Design review of the part built by this model. Coordinates are the model's own, in mm. Face numbers are marked on the shaded views. A direction names the side the tool comes from. Give positions to 0.01 mm unless a question says otherwise; leave off trailing zeros. Write each loop counter-clockwise with the first axis right and the second up, starting at its lowest first coordinate (ties: lowest second). Pieces come first, ordered by that corner, then holes. Notation, with made-up numbers: (29, 69) -> (60, 69) arc R13 cw to (60, 88) -> close; hole circle Ø3 at (23, -39). An arc over 180 degrees is marked (long way). Answer as a JSON object with one key per item and string values.
```python
from build123d import *

# Parameters (mm, degrees)
SKETCH_1_W               = 64
SKETCH_1_H               = 170
EXTRUDE_1_DEPTH          = 35
SKETCH_3_W               = 32.5
SKETCH_3_H               = 35
CUT_EXTRUDE_1_DEPTH      = 30
SKETCH_4_W               = 32.5
SKETCH_4_H               = 35
CUT_EXTRUDE_2_DEPTH      = 30
CUT_EXTRUDE_3_DEPTH      = 98.334474879
CUT_EXTRUDE_3_DEPTH_BACK = 98.334474879
SKETCH_5_R               = 5.5


with BuildPart() as part:
    # 草图1 → 凸台-拉伸1 (new body)
    with BuildSketch(Plane.XY):
        Rectangle(SKETCH_1_W, SKETCH_1_H)
    extrude(amount=EXTRUDE_1_DEPTH)

    # 草图3 → 切除-拉伸1 (cut)
    with BuildSketch(Plane.XY.offset(35)):
        with Locations((15.75, 67.5)):
            Rectangle(SKETCH_3_W, SKETCH_3_H)
        with Locations((15.75, -67.5)):
            Rectangle(SKETCH_3_W, SKETCH_3_H)
    extrude(amount=-CUT_EXTRUDE_1_DEPTH, mode=Mode.SUBTRACT)

    # 草图4 → 切除-拉伸2 (cut)
    with BuildSketch(Plane(origin=(0, 0, 0), x_dir=(-1, 0, 0), z_dir=(0, 0, -1))):
        with Locations((15.75, 67.5)):
            Rectangle(SKETCH_4_W, SKETCH_4_H)
        with Locations((15.75, -67.5)):
            Rectangle(SKETCH_4_W, SKETCH_4_H)
    extrude(amount=-CUT_EXTRUDE_2_DEPTH, mode=Mode.SUBTRACT)

    # 草图5 → 切除-拉伸3 (cut, two sides: drawn at the far end of the back side and taken through both)
    with BuildSketch(Plane.XY.offset(35).offset(-CUT_EXTRUDE_3_DEPTH_BACK)):
        with Locations((-18, 75)):
            Circle(SKETCH_5_R)
        with Locations((18, 75)):
            Circle(SKETCH_5_R)
        with Locations((18, -75)):
            Circle(SKETCH_5_R)
        with Locations((-18, -75)):
            Circle(SKETCH_5_R)
    extrude(amount=CUT_EXTRUDE_3_DEPTH + CUT_EXTRUDE_3_DEPTH_BACK, mode=Mode.SUBTRACT)


solid = part.part
```
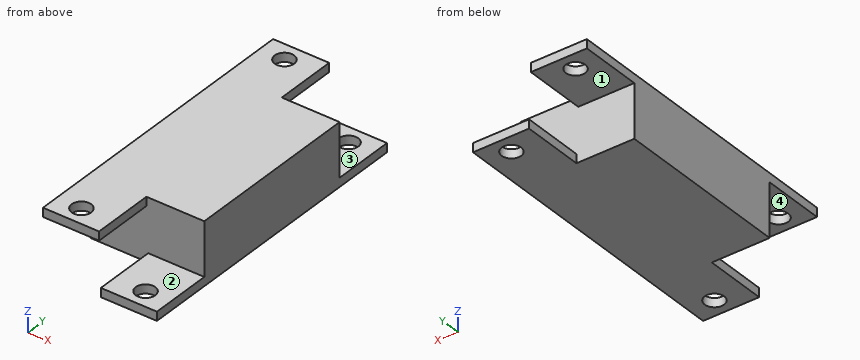
(1) We need section A-A, the plane y = -75. State the section outline as (x, z) points, then the cut area to 3 significant figures.
Here are the results:
{"outline": "(-32, 30) -> (-23.5, 30) -> (-23.5, 35) -> (-32, 35) -> close; (-12.5, 30) -> (-0.5, 30) -> (-0.5, 35) -> (-12.5, 35) -> close; (0.5, 0) -> (12.5, 0) -> (12.5, 5) -> (0.5, 5) -> close; (23.5, 0) -> (32, 0) -> (32, 5) -> (23.5, 5) -> close", "area": "205 mm²"}
(2) Clearance check with flat-ended pins moving along their axes: pin 1 (5 mm diameter, centred on x = 0.5, z = 10.5, fed in from -Y); pin 2 (16 mm diameter, centred on x = 10, y = -73.5, fed in from +Z); pin 3 (5.5 mm diameter, centred on y = 76, z = 33.5, fed in from +X). State where each tip first meets the part, or that it passes through.
Here are the results:
{"pin 1": "stops at y = -50", "pin 2": "stops at z = 5", "pin 3": "stops at x = -0.5"}
(3) We need section B-B, the plane x = 18. State the section outline as (y, z) points.
Here are the results:
{"outline": "(-85, 0) -> (-80.5, 0) -> (-80.5, 5) -> (-85, 5) -> close; (-69.5, 0) -> (69.5, 0) -> (69.5, 5) -> (50, 5) -> (50, 35) -> (-50, 35) -> (-50, 5) -> (-69.5, 5) -> close; (80.5, 0) -> (85, 0) -> (85, 5) -> (80.5, 5) -> close"}
(4) We need section D-D, the plane z = 8.5. State the section outline as (x, y) points.
Here are the results:
{"outline": "(-32, -50) -> (32, -50) -> (32, 50) -> (-32, 50) -> close"}
(5) We need section C-C, the plane x = -9. State the section outline as (y, z) points.
Here are the results:
{"outline": "(-85, 30) -> (-50, 30) -> (-50, 0) -> (50, 0) -> (50, 30) -> (85, 30) -> (85, 35) -> (-85, 35) -> close"}
(6) For the marked faces 1, 2, 3 and 4, list the 3-axis set-ups (+Z, -Z, +X, -X, +Y, -Y) from which the entire face can be reached by the end or side of a thin tool; tool diameter is ignored.
Here are the results:
{"face 1": "-Z, +X, -X, +Y", "face 2": "+Z, +X, -X, -Y", "face 3": "+Z, +X, -X, +Y", "face 4": "-Z, +X, -X, -Y"}
(7) For line 1 along Y through (x, z) = (18, 1.6); line 2 along X through (y, z) = (-75, 1.3); line 3 along Z through (x, y) = (19, 55), list the stretches that pass through material, from the lowest coordinate up.
Here are the results:
{"line 1": "y = -85 to -80.5, -69.5 to 69.5, 80.5 to 85", "line 2": "x = 0.5 to 12.5, 23.5 to 32", "line 3": "z = 0 to 5"}
